The listing builds one solid part. Answer for the finished solid, in the listing's coordinates (mm). A direction names the side the tool comes from. Coordinates: 2 decimals unless noted, no trailing zeros. Loops run counter-clockwise (first coordinate to the right, second up) from the corner with the lowest first, then second, coordinate; pieces in that order, holes last. Notation, with made-up numbers: (-1, 83.5) - (52, 83.5) arc R15 cw to (52, 103.5) - close; hole circle Ø10 at (75, 36.25). An arc over 180 degrees is marked (long way). Put each result on its own line as item: value.
```python
from build123d import *

# Parameters (mm, degrees)
F_100_X_50_X_5_1_DEPTH = 1150
CUT_EXTRUDE_1_REACH    = 1159.854


with BuildPart() as part:
    # Sketch11 → 矩形管 100 X 50 X 5(1) (new body)
    with BuildSketch(Plane(origin=(0, 0, 0), x_dir=(0, 0, -1), z_dir=(1, 0, 0))):
        with BuildLine():
            Line((-15, -50), (15, -50))
            ThreePointArc((15, -50), (22.071067812, -47.071067812), (25, -40))
            Line((25, -40), (25, 40))
            ThreePointArc((25, 40), (22.071067812, 47.071067812), (15, 50))
            Line((15, 50), (-15, 50))
            ThreePointArc((-15, 50), (-22.071067812, 47.071067812), (-25, 40))
            Line((-25, 40), (-25, -40))
            ThreePointArc((-25, -40), (-22.071067812, -47.071067812), (-15, -50))
        make_face()
        with BuildLine():
            Line((-15, -45), (15, -45))
            ThreePointArc((15, -45), (18.535533906, -43.535533906), (20, -40))
            Line((20, -40), (20, 40))
            ThreePointArc((20, 40), (18.535533906, 43.535533906), (15, 45))
            Line((15, 45), (-15, 45))
            ThreePointArc((-15, 45), (-18.535533906, 43.535533906), (-20, 40))
            Line((-20, 40), (-20, -40))
            ThreePointArc((-20, -40), (-18.535533906, -43.535533906), (-15, -45))
        make_face(mode=Mode.SUBTRACT)
    extrude(amount=F_100_X_50_X_5_1_DEPTH)

    # 切除-拉伸1: up to this face of the body (flat: up to its plane)
    cut_extrude_1_end = Plane(part.part.faces().sort_by_distance((575, 0, -25))[0])
    # 草图2 → 切除-拉伸1 (cut, up to the picked face)
    with BuildSketch(Plane(origin=(0, 75, 25), x_dir=(1, 0, 0), z_dir=(0, 0, 1)), mode=Mode.PRIVATE) as cut_extrude_1_sk1:
        Polygon((0, -25), (100, -125), (0, -125), align=None)
    cut_extrude_1_tool1 = split(extrude(cut_extrude_1_sk1.sketch, amount=-CUT_EXTRUDE_1_REACH, mode=Mode.PRIVATE), bisect_by=cut_extrude_1_end, keep=Keep.BOTH, mode=Mode.PRIVATE)
    # 草图2 → 切除-拉伸1 (cut, up to the picked face)
    with BuildSketch(Plane(origin=(0, 75, 25), x_dir=(1, 0, 0), z_dir=(0, 0, 1)), mode=Mode.PRIVATE) as cut_extrude_1_sk2:
        Polygon((1150, -71.913421349), (1103.086578651, -25), (1150, -25), align=None)
    cut_extrude_1_tool2 = split(extrude(cut_extrude_1_sk2.sketch, amount=-CUT_EXTRUDE_1_REACH, mode=Mode.PRIVATE), bisect_by=cut_extrude_1_end, keep=Keep.BOTH, mode=Mode.PRIVATE)
    add(cut_extrude_1_tool1.solids().sort_by(Axis((33.333333, -16.666667, 25), (0, 0, -1)))[0], mode=Mode.SUBTRACT)
    add(cut_extrude_1_tool2.solids().sort_by(Axis((1134.362193, 34.362193, 25), (0, 0, -1)))[0], mode=Mode.SUBTRACT)


solid = part.part
```
1) For a pull along Y with two mould halves and no side action, classify faces 1 (the face through (618, -50, 0)), 2 (the face through (615, -45, 0)), 3 (the face through (544, 50, 0)) as pulls with the +Y half, pulls with the -Y half, needs draft (parallel to the pull), parting line crosses it, or undercut.
Found:
face 1: pulls with the -Y half
face 2: undercut
face 3: pulls with the +Y half
2) The part is cut by section A-A (z = -1.5). Give the vertices of the cut face in (x, y), and give its area (3 significant figures).
Found:
outline: (0, 50) - (5, 45) - (1108.09, 45) - (1103.09, 50) - close; (95, -45) - (100, -50) - (1150, -50) - (1150, -45) - close
area: 10,800 mm^2
3) This flat-tipped pin is pushed along its axis until it touches: pin 1 (6 mm diameter, centred on y = 16.5, z = -19, fed in from +X) (3 decimals). Where does it stop, or does it pass through?
Found:
pin 1: stops at x = 1139.415
4) For faces 4 (the face through (572, -1, -20)), 5 (the face through (572, -1, -25)), determine the directions among +Z, -Z, +X, -X, +Y, -Y from which every point of the face is accessible in a straight line to the end or side of a thin tool.
Found:
face 4: +X, -X
face 5: -Z, +X, -X, +Y, -Y
5) The part is cut by section B-B (x = 805). Give the vertices of the cut face in (y, z).
Found:
outline: (-50, -15) arc R10 ccw to (-40, -25) - (40, -25) arc R10 ccw to (50, -15) - (50, 15) arc R10 ccw to (40, 25) - (-40, 25) arc R10 ccw to (-50, 15) - close; hole (-45, -15) arc R5 ccw to (-40, -20) - (40, -20) arc R5 ccw to (45, -15) - (45, 15) arc R5 ccw to (40, 20) - (-40, 20) arc R5 ccw to (-45, 15) - close
6) Straight lines are drawn through the part: L1, parallel to Y at x = 814, z = 14; L2, parallel to Z at x = 501.5, y = 13; L3, parallel to Y at x = 897, z = 16. For each, find the intervals that lie inside material, in ascending order. Write a range as [from, to].
Found:
L1: y = [-50, -45], [45, 50]
L2: z = [-25, -20], [20, 25]
L3: y = [-49.95, -44.9], [44.9, 49.95]
7) The part is cut by section C-C (y = 26). Give the vertices of the cut face in (x, z), and give its area (3 significant figures).
Found:
outline: (24, -25) - (1127.09, -25) - (1127.09, -20) - (24, -20) - close; (24, 20) - (1127.09, 20) - (1127.09, 25) - (24, 25) - close
area: 11,000 mm^2
